The model under review builds one solid part; all positions refer to its coordinate system, in mm. Face numbers are marked on the shaded views. A direction names the side the tool comes from. Coordinates: 2 decimals unless noted, no trailing zeros. Order: outer loops, then holes, each group sorted by start corner. A loop starts at its lowest first (then second) coordinate and runs counter-clockwise, first axis right, second up. Notation, with made-up numbers: M 56.5,-36 L 95.5,-36 A18 cw 95.5,-19 Z; hole C 21,74.25 d3. An arc over 180 degrees is marked long. One line per item, written item: value.
```python
from build123d import *

# Parameters (mm, degrees)
CUT_EXTRUDE1_REACH = 143.55
SKETCH2_R          = 21
SKETCH3_R          = 26
CUT_EXTRUDE2_DEPTH = 15


with BuildPart() as part:
    # Sketch1 → Revolve1 (revolve)
    with BuildSketch(Plane.XY):
        with BuildLine():
            Line((-16, 0), (-16, 97.5))
            Line((-16, 97.5), (-11, 97.5))
            Line((-11, 97.5), (-5.071594443, 83.37187176))
            ThreePointArc((-5.071594443, 83.37187176), (0, 80), (5.071594443, 83.37187176))
            Line((5.071594443, 83.37187176), (11, 97.5))
            Line((11, 97.5), (16, 97.5))
            Line((16, 97.5), (16, 0))
            Line((16, 0), (-16, 0))
        make_face()
    revolve(axis=Axis((16, 0, 0), (-1, 0, 0)))

    # Sketch2 → Cut-Extrude1 (cut, up to next)
    with BuildSketch(Plane(origin=(16, 0, 0), x_dir=(0, 0, -1), z_dir=(1, 0, 0)), mode=Mode.PRIVATE) as cut_extrude1_sk1:
        with Locations(Location((0, 0, 0), (0, 0, 90))):
            Circle(SKETCH2_R)
    cut_extrude1_tool1 = extrude(cut_extrude1_sk1.sketch, amount=-CUT_EXTRUDE1_REACH, mode=Mode.PRIVATE) & part.part
    add(cut_extrude1_tool1.solids().sort_by_distance((16, 0, 0))[0], mode=Mode.SUBTRACT)

    # Sketch3 → Cut-Extrude2 (cut)
    with BuildSketch(Plane(origin=(16, 0, 0), x_dir=(0, 0, -1), z_dir=(1, 0, 0))):
        with Locations(Location((0, 0, 0), (0, 0, 90))):
            Circle(SKETCH3_R)
    cut_extrude2 = extrude(amount=-CUT_EXTRUDE2_DEPTH, mode=Mode.SUBTRACT)

    # Mirror1: Cut-Extrude2 across plane
    add(cut_extrude2.mirror(Plane(origin=(0, 0, 0), x_dir=(0, 0, 1), z_dir=(1, 0, 0))), mode=Mode.SUBTRACT)


solid = part.part
```
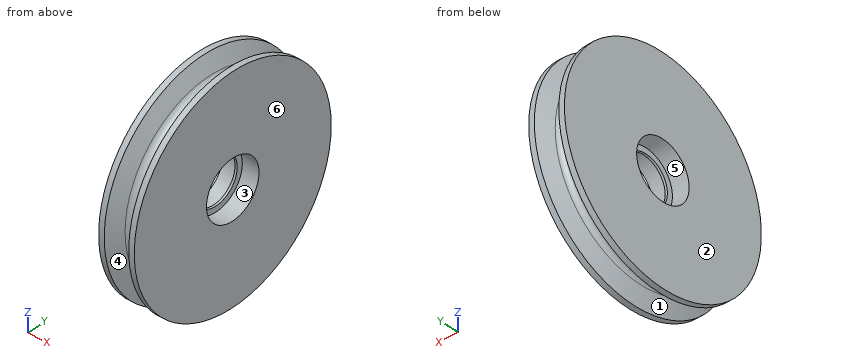
(1) Mouldability with a two-part tool opening along Y and no side actions: class the marked faces 1, 2 and 3 as +Y half, -Y half, draft (parallel to the pull), parting line (faces both ways), or undercut.
Geometry results:
face 1: parting line
face 2: draft
face 3: undercut
(2) We need section A-A, the plane z = 0. State the section outline as (x, y) points.
Geometry results:
outline: M -16,-97.5 L -11,-97.5 L -5.07,-83.37 A5.5 cw 5.07,-83.37 L 11,-97.5 L 16,-97.5 L 16,-26 L 1,-26 L 1,-21 L -1,-21 L -1,-26 L -16,-26 Z; M -16,26 L -1,26 L -1,21 L 1,21 L 1,26 L 16,26 L 16,97.5 L 11,97.5 L 5.07,83.37 A5.5 cw -5.07,83.37 L -11,97.5 L -16,97.5 Z
(3) Insertion check: pin 1 Ø12 at (x, y) = (-9, -54.5) entering from +Z; pin 2 Ø4 at (x, z) = (10.5, -50) entering from +Y; pin 3 Ø5 at (x, y) = (9, -23.5) entering from +Z; pin 4 Ø25 at (y, z) = (0, 0) entering from -X. Each pin has a flat end and moves straight along its axis. Give the tip position at first contact, or say it passes through.
Geometry results:
pin 1: stops at z = 84.38
pin 2: stops at y = 84.83
pin 3: stops at z = 94.99
pin 4: passes through
(4) Tool access review of the marked faces 4, 5 and 6: name each direction out of +Z, -Z, +X, -X, +Y, -Y from which nothing blocks a thin tool from reaching the whole face with its end or side.
Geometry results:
face 4: none
face 5: -X
face 6: +Z, -Z, +X, +Y, -Y
(5) For L1, parallel to Z at x = -9.5, y = 0; L2, parallel to X at y = -44, z = 77.5; L3, parallel to Z at x = 14, y = 15, list the stretches that pass through material, from the lowest coordinate up.
Geometry results:
L1: z = -93.93 to -26, 26 to 93.93
L2: x = -16 to -7.48, 7.48 to 16
L3: z = -96.34 to -21.24, 21.24 to 96.34
